```python
from build123d import *

# Parameters (mm, degrees)
SKETCH_1_R      = 50
SKETCH_1_R_2    = 2.25
EXTRUDE_1_DEPTH = 1
CHAMFER_1_SIZE  = 0.8


with BuildPart() as part:
    # 草图1 → 凸台-拉伸1 (new body)
    with BuildSketch(Plane.XY):
        Circle(SKETCH_1_R)
        with Locations((0, 15)):
            Circle(SKETCH_1_R_2, mode=Mode.SUBTRACT)
        with Locations((12.990381057, -7.5)):
            Circle(SKETCH_1_R_2, mode=Mode.SUBTRACT)
        with Locations((-12.990381057, -7.5)):
            Circle(SKETCH_1_R_2, mode=Mode.SUBTRACT)
    extrude(amount=EXTRUDE_1_DEPTH)

    # 倒角1
    chamfer_1_edges = [part.edges().sort_by_distance(p)[0] for p in [
        (-15.240381057, -7.5, 1),
        (-2.25, 15, 1),
        (10.740381057, -7.5, 1),
    ]]
    chamfer(chamfer_1_edges, length=CHAMFER_1_SIZE)


solid = part.part
```
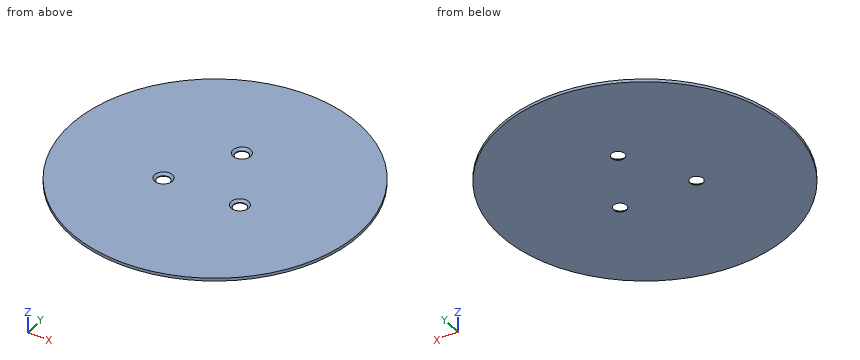
Can you work these out from the model? Positions are in its coordinate system, mm. Round coordinates to 2 decimals unless told otherwise and drop trailing zeros. Loops run counter-clockwise (first coordinate to the right, second up) from the corner with the lowest first, then second, coordinate; pieces in that order, holes last. Notation, with made-up numbers: M 49,44 L 96,44 A28 ccw 96,77 Z; hole C 76.25,-27 d9. An arc over 180 degrees is marked long. Answer as a JSON object with one key per item and string values. Group by question number.
Q1. Will these pins go through, and if not, where does the flat tip stop? pin 1 (5 mm diameter, centred on x = -12.99, y = -7.5, fed in from +Z); pin 2 (6 mm diameter, centred on x = 12.99, y = -7.5, fed in from +Z).
Q2. Imagine slicing it at D-D, the plane z = 0.45. Please give me the cut outline in (x, y).
Q3. Imagine slicing it at B-B, the plane y = -7.5. Please give me the cut outline in (x, z).
Q4. Imagine slicing it at C-C, the plane y = 15. Please give me the cut outline in (x, z), then the cut area to 3 significant figures.
Q5. Imagine slicing it at A-A, the plane x = 0. Please give me the cut outline in (y, z), then the cut area to 3 significant figures.
Q6. Please list where these lines run through material, in increasing order: L1, parallel to X at y = -7, z = 0.95; L2, parallel to Y at x = 0, z = 0.15; L3, parallel to X at y = -6, z = 0.25.
Findings:
{
 "1": {"pin 1": "stops at z = 0.45", "pin 2": "stops at z = 0.95"},
 "2": {"outline": "C 0,0 d100; hole C -12.99,-7.5 d5; hole C 0,15 d5; hole C 12.99,-7.5 d5"},
 "3": {"outline": "M -49.43,0 L -15.24,0 L -15.24,0.2 L -16.04,1 L -49.43,1 Z; M -10.74,0 L 10.74,0 L 10.74,0.2 L 9.94,1 L -9.94,1 L -10.74,0.2 Z; M 15.24,0 L 49.43,0 L 49.43,1 L 16.04,1 L 15.24,0.2 Z"},
 "4": {"outline": "M -47.7,0 L -2.25,0 L -2.25,0.2 L -3.05,1 L -47.7,1 Z; M 2.25,0 L 47.7,0 L 47.7,1 L 3.05,1 L 2.25,0.2 Z", "area": "90.3 mm2"},
 "5": {"outline": "M -50,0 L 12.75,0 L 12.75,0.2 L 11.95,1 L -50,1 Z; M 17.25,0 L 50,0 L 50,1 L 18.05,1 L 17.25,0.2 Z", "area": "94.9 mm2"},
 "6": {"L1": "x = -49.51 to -15.95, -10.03 to 10.03, 15.95 to 49.51", "L2": "y = -50 to 12.75, 17.25 to 50", "L3": "x = -49.64 to -14.73, -11.25 to 11.25, 14.73 to 49.64"}
}
